Work out the finished part from the listing and answer in its coordinate system (mm). Face numbers are marked on the shaded views. Round coordinates to 2 decimals unless told otherwise and drop trailing zeros. Order: outer loops, then holes, each group sorted by start corner. A loop starts at its lowest first (then second) coordinate and runs counter-clockwise, first axis right, second up. Notation, with made-up numbers: (53, 34.5) -> (104, 34.5) arc R31 cw to (104, 59.5) -> close; hole circle Ø1 at (17.5, -23). An arc over 180 degrees is marked (long way). Use a Markdown table: item, result. Add a question column.
Item 1: A cutting plane is placed at A-A, the plane y = 0. Determine the outline of the cut face in (x, z).
Item 2: A cutting plane is placed at C-C, the plane z = 13.25. Determine the outline of the cut face in (x, y).
Item 3: Flat-ended cylindrical pins translate along their axes: P1, Ø6, axis at x = 0, y = -2, coming from the -Z side; P2, Ø1, axis at x = 1.5, z = 6, coming from the +Y side; P3, Ø7, axis at x = 0, y = 0, coming from the -Z side. Find the tip coordinate at first contact, or state that the pin passes through.
Item 4: For a pull along X with two mould halves and no side action, classify the marked faces 1, 2, 3 and 4 as +X half, -X half, draft (parallel to the pull), parting line (faces both ways), or undercut.
Item 5: A cutting plane is placed at D-D, the plane z = 5.5. Determine the outline of the cut face in (x, y), plus the area to 3 significant figures.
Item 6: Find the intervals of material crossed by L1, parallel to Y at x = 0, z = 13.2; L2, parallel to Y at x = 0, z = 8; L3, parallel to X at y = 0.5, z = 11.75, in increasing order. Write a range as [from, to].
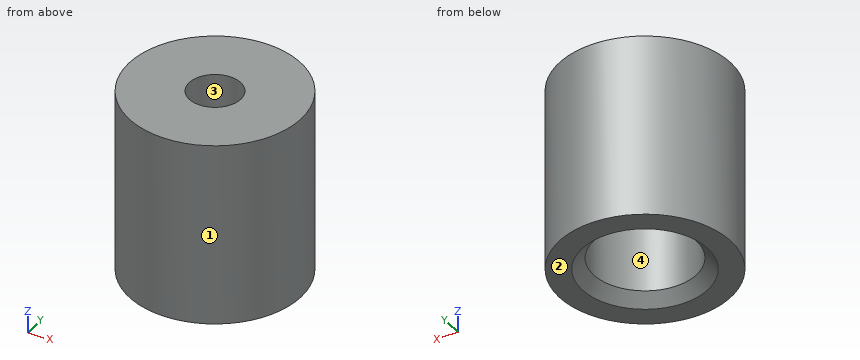
from build123d import *

# Parameters (mm, degrees)
SKETCH_1_R                   = 7.5
EXTRUDE_1_DEPTH              = 16
HOLE_WIZARD_M4_1_D           = 4.5
HOLE_WIZARD_M4_1_CBORE_D     = 9
HOLE_WIZARD_M4_1_CBORE_DEPTH = 12
CHAMFER_1_SIZE               = 1


with BuildPart() as part:
    # 草图1 → 凸台-拉伸1 (new body)
    with BuildSketch(Plane.XY):
        Circle(SKETCH_1_R)
    extrude(amount=EXTRUDE_1_DEPTH)

    # M4 六角凹头螺钉的柱形沉头孔1 (through all)
    with Locations(Plane(origin=(0, 0, 0), x_dir=(-1, 0, 0), z_dir=(0, 0, -1))):
        with Locations((0, 0)):
            CounterBoreHole(HOLE_WIZARD_M4_1_D / 2, HOLE_WIZARD_M4_1_CBORE_D / 2, HOLE_WIZARD_M4_1_CBORE_DEPTH)

    # 倒角1
    chamfer_1_edges = [part.edges().sort_by_distance(p)[0] for p in [
        (4.5, 0, 0),
    ]]
    chamfer(chamfer_1_edges, length=CHAMFER_1_SIZE)


solid = part.part
Reported:
| question | item | result |
|---|---|---|
| 1 | outline | (-7.5, 0) -> (-5.5, 0) -> (-4.5, 1) -> (-4.5, 12) -> (-2.25, 12) -> (-2.25, 16) -> (-7.5, 16) -> close; (2.25, 12) -> (4.5, 12) -> (4.5, 1) -> (5.5, 0) -> (7.5, 0) -> (7.5, 16) -> (2.25, 16) -> close |
| 2 | outline | circle Ø15 at (0, 0); hole circle Ø4.5 at (0, 0) |
| 3 | P1 | z = 0.5 |
| 3 | P2 | y = 7.43 |
| 3 | P3 | z = 12 |
| 4 | face 1 | parting line |
| 4 | face 2 | draft |
| 4 | face 3 | undercut |
| 4 | face 4 | undercut |
| 5 | outline | circle Ø15 at (0, 0); hole circle Ø9 at (0, 0) |
| 5 | area | 113 mm² |
| 6 | L1 | [-7.5, -2.25], [2.25, 7.5] |
| 6 | L2 | [-7.5, -4.5], [4.5, 7.5] |
| 6 | L3 | [-7.48, -4.47], [4.47, 7.48] |
